from build123d import *

# Parameters (mm, degrees)
SKETCH1_W           = 12.7
SKETCH1_H           = 12.7
SKETCH1_R           = 1.25
BOSS_EXTRUDE1_DEPTH = 2
CHAMFER1_SIZE       = 1
SKETCH2_R           = 2.7
BOSS_EXTRUDE2_DEPTH = 4.6
SKETCH3_R           = 2.7
BOSS_EXTRUDE3_DEPTH = 5.2


with BuildPart() as part:
    # Sketch1 → Boss-Extrude1 (new body)
    with BuildSketch(Plane.XY):
        with Locations((-6.35, -6.35)):
            Rectangle(SKETCH1_W, SKETCH1_H)
        with Locations((-10.65, -2.05)):
            Circle(SKETCH1_R, mode=Mode.SUBTRACT)
        with Locations((-2.05, -2.05)):
            Circle(SKETCH1_R, mode=Mode.SUBTRACT)
        with Locations(Location((-2.05, -10.65, 0), (0, 0, 180))):
            Circle(SKETCH1_R, mode=Mode.SUBTRACT)
        with Locations(Location((-10.65, -10.65, 0), (0, 0, 180))):
            Circle(SKETCH1_R, mode=Mode.SUBTRACT)
    extrude(amount=BOSS_EXTRUDE1_DEPTH)

    # Chamfer1
    chamfer1_edges = [part.edges().sort_by_distance(p)[0] for p in [
        (0, -12.7, 1),
        (-12.7, -12.7, 1),
        (-12.7, 0, 1),
        (0, 0, 1),
    ]]
    chamfer(chamfer1_edges, length=CHAMFER1_SIZE)

    # Sketch2 → Boss-Extrude2 (add)
    with BuildSketch(Plane.XY.offset(2)):
        with Locations((-6.35, -6.35)):
            Circle(SKETCH2_R)
    extrude(amount=BOSS_EXTRUDE2_DEPTH)

    # Sketch3 → Boss-Extrude3 (add)
    with BuildSketch(Plane.XY.offset(6.6)):
        with Locations((-6.35, -6.35)):
            Circle(SKETCH3_R)
    extrude(amount=BOSS_EXTRUDE3_DEPTH)


solid = part.part
Here's how the part is built. I have some questions about the finished solid (model axes, mm). A direction names the side the tool comes from. Give positions to 0.01 mm unless a question says otherwise; leave off trailing zeros. Order: outer loops, then holes, each group sorted by start corner. A loop starts at its lowest first (then second) coordinate and runs counter-clockwise, first axis right, second up. Notation, with made-up numbers: M -21.5,11.25 L -5.5,11.25 A26 ccw -5.5,29.25 Z; hole C 0.25,-9.75 d1. An arc over 180 degrees is marked long. Answer as a JSON object with one key per item and string values. Group by question number.
1) Suppose I cut it at B-B, the plane x = -2.05. Write out the boundary of the cut face in (y, z).
2) Suppose I cut it at C-C, the plane y = -6.35. Write out the boundary of the cut face in (x, z).
3) We'd pull the mould along X, two halves only. Please class faces 3 (the flat face through (-6, -12.7, 1)), 4 (the cylindrical face through (-11.227, -9.541, 0.986)), 5 (the flat face through (-0.5, -12.2, 1)): pulls with the +X half, pulls with the -X half, needs draft (parallel to the pull), parting line crosses it, or undercut.
4) I'm going to push flat-ended pins straight in: pin 1 Ø2 at (x, y) = (-10, -8.5) entering from +Z; pin 2 Ø2 at (x, z) = (-4, 5) entering from -Y; pin 3 Ø5 at (x, z) = (-2, 9) entering from -Y. Where does each tip first touch, or does it pass through?
5) Please list where these lines run through material, in increasing order: L1, parallel to Y at x = -10.65, z = 1.3; L2, parallel to Y at x = -9.75, z = 1; L3, parallel to Z at x = -2, y = -5. Write a range as [from, to].
6) Suppose I cut it at A-A, the plane y = -11. Write out the boundary of the cut face in (x, z).
7) On a 3-axis mill with a long thin cutter (end or side, diameter ignored), from which of +Z, -Z, +X, -X, +Y, -Y can I reach the whole of each face in a straight line? I mean faces 1 (the cylindrical face through (-3.775, -5.539, 6.831)), 2 (the flat face through (-6, 0, 1)). Say none if no direction works.
Results found:
{
 "1": {"outline": "M -12.7,0 L -11.9,0 L -11.9,2 L -12.7,2 Z; M -9.4,0 L -3.3,0 L -3.3,2 L -9.4,2 Z; M -0.8,0 L 0,0 L 0,2 L -0.8,2 Z"},
 "2": {"outline": "M -12.7,0 L 0,0 L 0,2 L -3.65,2 L -3.65,11.8 L -9.05,11.8 L -9.05,2 L -12.7,2 Z"},
 "3": {"face 3": "needs draft", "face 4": "undercut", "face 5": "pulls with the +X half"},
 "4": {"pin 1": "z = 2", "pin 2": "y = -8.69", "pin 3": "y = -8.32"},
 "5": {"L1": "[-12.7, -11.9], [-9.4, -3.3], [-0.8, 0]", "L2": "[-12.7, -11.52], [-9.78, -2.92], [-1.18, 0]", "L3": "[0, 2]"},
 "6": {"outline": "M -12.7,0 L -11.85,0 L -11.85,2 L -12.7,2 Z; M -9.45,0 L -3.25,0 L -3.25,2 L -9.45,2 Z; M -0.85,0 L 0,0 L 0,2 L -0.85,2 Z"},
 "7": {"face 1": "+Z", "face 2": "+Z, -Z, +X, -X, +Y"}
}
